Build history of the part. All positions in model axes, mm. Face numbers are marked on the shaded views. Give positions to 0.01 mm unless a question says otherwise; leave off trailing zeros. Write each loop counter-clockwise with the first axis right and the second up, starting at its lowest first coordinate (ties: lowest second). Pieces come first, ordered by that corner, then holes. Notation, with made-up numbers: (-21.75, -26.5) -> (33.25, -26.5) arc R37 ccw to (33.25, 11.5) -> close; hole circle Ø1 at (7.5, 0.25). An arc over 180 degrees is marked (long way). Write item = value, one per line. Start each with the question number.
Q1. Mould opens along X. For the marked faces 1, 2, 3 and 4 say: pulls with the +X half, pulls with the -X half, needs draft (parallel to the pull), parting line crosses it, or undercut.
Q2. Saw through at A-A, the plane y = 5. List the corners of the cut face in (x, z).
Q3. Saw through at C-C, the plane z = 4.5. List the corners of the cut face in (x, y).
Q4. Wall check: line 1 (Y direction, x = 12.5, z = 3.5); line 2 (Y direction, x = 0, z = 4.5); line 3 (X direction, y = 3.5, z = 3.75). Give the ranges that are in metal, low to high.
Q5. Saw through at B-B, the plane x = -12.5. List the corners of the cut face in (y, z).
Q6. Drop a flat-ended pin along its axis: P1, Ø5.5, axis at x = 0, y = -5, coming from the +Z side. Give the stop position or say it passes through.
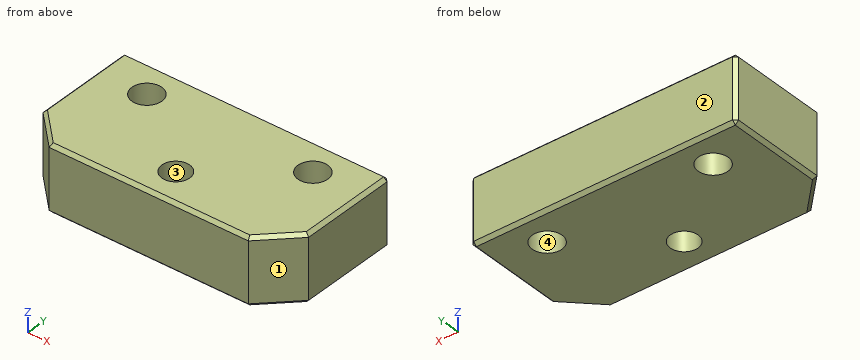
from build123d import *

# Parameters (mm, degrees)
SKETCH_1_W              = 40
SKETCH_1_H              = 20
EXTRUDE_1_DEPTH         = 10
HOLE_WIZARD_4_5_4_5_1_D = 4.5
HOLE_WIZARD_M5_1_D      = 4.2
CHAMFER_1_SIZE          = 5
CHAMFER_2_SIZE          = 0.5


with BuildPart() as part:
    # 草图1 → 凸台-拉伸1 (new body)
    with BuildSketch(Plane.XY):
        Rectangle(SKETCH_1_W, SKETCH_1_H)
    extrude(amount=EXTRUDE_1_DEPTH)

    # Ø4.5 (4.5) 直径孔1 (through all)
    with Locations(Plane.XY.offset(10)):
        with Locations((12.5, 5), (-12.5, 5)):
            Hole(HOLE_WIZARD_4_5_4_5_1_D / 2)

    # M5 螺纹孔1 (through all)
    with Locations(Plane.XY.offset(10)):
        with Locations((0, -5)):
            Hole(HOLE_WIZARD_M5_1_D / 2)

    # 倒角1
    chamfer_1_edges = [part.edges().sort_by_distance(p)[0] for p in [
        (20, -10, 5),
        (-20, -10, 5),
    ]]
    chamfer(chamfer_1_edges, length=CHAMFER_1_SIZE)

    # 倒角2
    chamfer_2_edges = [part.edges().sort_by_distance(p)[0] for p in [
        (-20, 2.5, 10),
        (0, -10, 0),
        (0, -10, 10),
        (20, 2.5, 0),
        (17.5, -7.5, 0),
        (-17.5, -7.5, 0),
        (20, 2.5, 10),
        (17.5, -7.5, 10),
        (-17.5, -7.5, 10),
        (-20, 2.5, 0),
        (0, 10, 0),
        (-20, 10, 5),
        (20, 10, 5),
        (0, 10, 10),
    ]]
    chamfer(chamfer_2_edges, length=CHAMFER_2_SIZE)


solid = part.part
Report:
q1.face_1 = pulls with the +X half
q1.face_2 = needs draft
q1.face_3 = undercut
q1.face_4 = undercut
q2.outline = (-20, 0.5) -> (-19.5, 0) -> (-14.75, 0) -> (-14.75, 10) -> (-19.5, 10) -> (-20, 9.5) -> close; (-10.25, 0) -> (10.25, 0) -> (10.25, 10) -> (-10.25, 10) -> close; (14.75, 0) -> (19.5, 0) -> (20, 0.5) -> (20, 9.5) -> (19.5, 10) -> (14.75, 10) -> close
q3.outline = (-20, -5) -> (-15, -10) -> (15, -10) -> (20, -5) -> (20, 9.5) -> (19.5, 10) -> (-19.5, 10) -> (-20, 9.5) -> close; hole circle Ø4.5 at (-12.5, 5); hole circle Ø4.2 at (0, -5); hole circle Ø4.5 at (12.5, 5)
q4.line_1 = -10 to 2.75, 7.25 to 10
q4.line_2 = -10 to -7.1, -2.9 to 10
q4.line_3 = -20 to -14.18, -10.82 to 10.82, 14.18 to 20
q5.outline = (-10, 0.5) -> (-9.5, 0) -> (2.75, 0) -> (2.75, 10) -> (-9.5, 10) -> (-10, 9.5) -> close; (7.25, 0) -> (9.5, 0) -> (10, 0.5) -> (10, 9.5) -> (9.5, 10) -> (7.25, 10) -> close
q6.P1 = 10
